Here's how the part is built. I have some questions about the finished solid (model axes, mm). A direction names the side the tool comes from. Coordinates: 2 decimals unless noted, no trailing zeros. Loops run counter-clockwise (first coordinate to the right, second up) from the corner with the lowest first, then second, coordinate; pieces in that order, holes last. Notation, with made-up numbers: (31, 41) - (88, 41) arc R16 ccw to (88, 54) - close; hole circle Ø3 at (6, 52). An arc over 180 degrees is marked (long way). Use a Markdown table: item, result.
```python
from build123d import *

# Parameters (mm, degrees)
SKETCH_1_W              = 47
SKETCH_1_H              = 43
EXTRUDE_1_DEPTH         = 36
SKETCH_2_W              = 37.2
SKETCH_2_H              = 43
CUT_EXTRUDE_1_DEPTH     = 28
CUT_EXTRUDE_2_REACH     = 64.986
SKETCH_3_R              = 2
SKETCH_4_W              = 37.2
SKETCH_4_H              = 6
EXTRUDE_2_DEPTH         = 28
FILLET_1_R              = 3
CUT_EXTRUDE_3_REACH     = 51.482
SKETCH_5_R              = 4
HOLE_WIZARD_M3_1_REACH  = 50.068
HOLE_WIZARD_M3_1_BORE_R = 1.25
HOLE_WIZARD_M3_2_REACH  = 57.419
HOLE_WIZARD_M3_2_BORE_R = 1.25
SKETCH_8_W              = 25
SKETCH_8_H              = 9.5
EXTRUDE_3_DEPTH         = 8
SKETCH_9_R              = 2.5
CUT_EXTRUDE_4_DEPTH     = 14


with BuildPart() as part:
    # 草图1 → 凸台-拉伸1 (new body)
    with BuildSketch(Plane.XY):
        Rectangle(SKETCH_1_W, SKETCH_1_H)
    extrude(amount=EXTRUDE_1_DEPTH)

    # 草图2 → 切除-拉伸1 (cut)
    with BuildSketch(Plane.XY.offset(36)):
        Rectangle(SKETCH_2_W, SKETCH_2_H)
    extrude(amount=-CUT_EXTRUDE_1_DEPTH, mode=Mode.SUBTRACT)

    # 切除-拉伸2: up to this face of the body (flat: up to its plane)
    cut_extrude_2_end = Plane(part.part.faces().sort_by_distance((23.5, 0, 18))[0])
    # 草图3 → 切除-拉伸2 (cut, up to the picked face)
    with BuildSketch(Plane.ZY.offset(23.5), mode=Mode.PRIVATE) as cut_extrude_2_sk1:
        with Locations((32, 13.5)):
            Circle(SKETCH_3_R)
    cut_extrude_2_tool1 = split(extrude(cut_extrude_2_sk1.sketch, amount=-CUT_EXTRUDE_2_REACH, mode=Mode.PRIVATE), bisect_by=cut_extrude_2_end, keep=Keep.BOTH, mode=Mode.PRIVATE)
    # 草图3 → 切除-拉伸2 (cut, up to the picked face)
    with BuildSketch(Plane.ZY.offset(23.5), mode=Mode.PRIVATE) as cut_extrude_2_sk2:
        with Locations((32, -13.5)):
            Circle(SKETCH_3_R)
    cut_extrude_2_tool2 = split(extrude(cut_extrude_2_sk2.sketch, amount=-CUT_EXTRUDE_2_REACH, mode=Mode.PRIVATE), bisect_by=cut_extrude_2_end, keep=Keep.BOTH, mode=Mode.PRIVATE)
    add(cut_extrude_2_tool1.solids().sort_by(Axis((-23.5, 13.5, 32), (1, 0, 0)))[0], mode=Mode.SUBTRACT)
    add(cut_extrude_2_tool2.solids().sort_by(Axis((-23.5, -13.5, 32), (1, 0, 0)))[0], mode=Mode.SUBTRACT)

    # 草图4 → 凸台-拉伸2 (add)
    with BuildSketch(Plane.XY.offset(8)):
        Rectangle(SKETCH_4_W, SKETCH_4_H)
    extrude(amount=EXTRUDE_2_DEPTH)

    # 圆角1
    fillet_1_edges = [part.edges().sort_by_distance(p)[0] for p in [
        (18.6, -12.25, 8),
        (-18.6, 12.25, 8),
        (18.6, 12.25, 8),
        (-18.6, -12.25, 8),
    ]]
    fillet(fillet_1_edges, radius=FILLET_1_R)

    # 草图5 → 切除-拉伸3 (cut, up to next)
    with BuildSketch(Plane(origin=(0, 3, 0), x_dir=(1, 0, 0), z_dir=(0, 1, 0)), mode=Mode.PRIVATE) as cut_extrude_3_sk1:
        with Locations(Location((0, -20, 0), (0, 0, 270))):
            Circle(SKETCH_5_R)
    cut_extrude_3_tool1 = extrude(cut_extrude_3_sk1.sketch, amount=-CUT_EXTRUDE_3_REACH, mode=Mode.PRIVATE) & part.part
    add(cut_extrude_3_tool1.solids().sort_by_distance((0, 3, 20))[0], mode=Mode.SUBTRACT)

    # M3 螺纹孔1 bore (on position points) → M3 螺纹孔1 (cut, up to next)
    with BuildSketch(Plane.XY.offset(36), mode=Mode.PRIVATE) as hole_wizard_m3_1_sk1:
        Circle(HOLE_WIZARD_M3_1_BORE_R)
    hole_wizard_m3_1_tool1 = extrude(hole_wizard_m3_1_sk1.sketch, amount=-HOLE_WIZARD_M3_1_REACH, mode=Mode.PRIVATE) & part.part
    add(hole_wizard_m3_1_tool1.solids().sort_by_distance((0, 0, 36))[0], mode=Mode.SUBTRACT)

    # M3 螺纹孔2 bore (on position points) → M3 螺纹孔2 (cut, up to next)
    with BuildSketch(Plane(origin=(-23.5, 0, 20), x_dir=(0, 0, -1), z_dir=(-1, 0, 0)), mode=Mode.PRIVATE) as hole_wizard_m3_2_sk1:
        Circle(HOLE_WIZARD_M3_2_BORE_R)
    hole_wizard_m3_2_tool1 = extrude(hole_wizard_m3_2_sk1.sketch, amount=-HOLE_WIZARD_M3_2_REACH, mode=Mode.PRIVATE) & part.part
    add(hole_wizard_m3_2_tool1.solids().sort_by_distance((-23.5, 0, 20))[0], mode=Mode.SUBTRACT)

    # 草图8 → 凸台-拉伸3 (add)
    with BuildSketch(Plane(origin=(0, 0, 0), x_dir=(-1, 0, 0), z_dir=(0, 0, -1))):
        with Locations((0, 26.25)):
            Rectangle(SKETCH_8_W, SKETCH_8_H)
        with Locations((0, -26.25)):
            Rectangle(SKETCH_8_W, SKETCH_8_H)
    extrude(amount=-EXTRUDE_3_DEPTH)

    # 草图9 → 切除-拉伸4 (cut)
    with BuildSketch(Plane.ZY.offset(23.5)):
        with Locations((20, 0)):
            Circle(SKETCH_9_R)
    extrude(amount=-CUT_EXTRUDE_4_DEPTH, mode=Mode.SUBTRACT)


solid = part.part
```
Q1. I want a section at B-B, the plane y = -13.5. Write out the boundary of the cut face in (x, z), then the cut area to 3 significant figures.
Check values:
| item | result |
|---|---|
| outline | (-23.5, 0) - (23.5, 0) - (23.5, 30) - (18.6, 30) - (18.6, 11) arc R3 cw to (15.6, 8) - (-15.6, 8) arc R3 cw to (-18.6, 11) - (-18.6, 30) - (-23.5, 30) - close; (-23.5, 34) - (-18.6, 34) - (-18.6, 36) - (-23.5, 36) - close; (18.6, 34) - (23.5, 34) - (23.5, 36) - (18.6, 36) - close |
| area | 615 mm^2 |
Q2. Will these pins go through, and if not, where does the flat tip stop? P1, Ø4, axis at x = 7, y = -23.5, coming from the +Z side; P2, Ø8.5, axis at x = 4.5, z = 26, coming from the -Y side; P3, Ø5.5, axis at x = 20.5, z = 25, coming from the +Y side; P4, Ø3, axis at y = -13.5, z = 32, coming from the +X side.
Check values:
| item | result |
|---|---|
| P1 | z = 8 |
| P2 | y = -3 |
| P3 | y = 21.5 |
| P4 | through |
Q3. If we mould it in two halves opening along X, with no side actions, what happens to faces 6 (the face through (-12.5, 26, 4)), 7 (the face through (23.5, 0, 18)), 8 (the face through (-17.74, 12.38, 8.9)), 9 (the face through (-6.687, 0.479, 18.845))? For each: pulls with the +X half, pulls with the -X half, needs draft (parallel to the pull), parting line crosses it, or undercut.
Check values:
| item | result |
|---|---|
| face 6 | pulls with the -X half |
| face 7 | pulls with the +X half |
| face 8 | undercut |
| face 9 | needs draft |
Q4. I want a section at C-C, the plane x = 0. Write out the boundary of the cut face in (y, z).
Check values:
| item | result |
|---|---|
| outline | (-31, 0) - (31, 0) - (31, 8) - (3, 8) - (3, 16) - (-3, 16) - (-3, 8) - (-31, 8) - close; (-3, 24) - (-1.25, 24) - (-1.25, 36) - (-3, 36) - close; (1.25, 24) - (3, 24) - (3, 36) - (1.25, 36) - close |
Q5. Please list where these lines run through material, in increasing order: L1, parallel to Y at x = 21.6, z = 32; L2, parallel to X at y = -5.5, z = 32.5; L3, parallel to Y at x = 0, z = 26.75. Write a range as from..to.
Check values:
| item | result |
|---|---|
| L1 | -21.5..-15.5, -11.5..11.5, 15.5..21.5 |
| L2 | -23.5..-18.6, 18.6..23.5 |
| L3 | -3..-1.25, 1.25..3 |
Q6. I want a section at D-D, the plane z = 26. Write out the boundary of the cut face in (x, y).
Check values:
| item | result |
|---|---|
| outline | (-23.5, -21.5) - (-18.6, -21.5) - (-18.6, -3) - (18.6, -3) - (18.6, -21.5) - (23.5, -21.5) - (23.5, 21.5) - (18.6, 21.5) - (18.6, 3) - (-18.6, 3) - (-18.6, 21.5) - (-23.5, 21.5) - close; hole circle Ø2.5 at (0, 0) |
Q7. I want a section at A-A, the plane z = 32. Give the number of separate pieces and of enclosed holes in the cut face, then the cut area to 3 significant figures.
Check values:
| item | result |
|---|---|
| separate pieces | 5 |
| enclosed holes | 1 |
| area | 561 mm^2 |
Q8. Which directions (+Z, -Z, +X, -X, +Y, -Y) give clear straight access to the entire face, cutting with the end or side of a thin tool? Please do faces 1 (the face through (20, -21.5, 14)), 2 (the face through (20, 21.5, 14)), 3 (the face through (-21, 21.5, 14)), 4 (the face through (-0.27, -1.22, 29.98)), 5 (the face through (0, 17, 8)).
Check values:
| item | result |
|---|---|
| face 1 | +Z, -Z, +X, -Y |
| face 2 | +Z, -Z, +X, +Y |
| face 3 | +Z, -Z, -X, +Y |
| face 4 | +Z |
| face 5 | +Z, +Y |
